CAD build for the part. Positions are in the model's coordinates, mm. A direction names the side the tool comes from. Coordinates: 2 decimals unless noted, no trailing zeros. Write each question's results on one line, items separated by ' | '.
from build123d import *

# Parameters (mm, degrees)
EXTRUDE_1_DEPTH     = 3
SKETCH_7_R          = 1
CUT_EXTRUDE_2_DEPTH = 6.5
FILLET_3_R          = 1
CUT_EXTRUDE_START   = -43.5
SKETCH_8_R          = 1.5
CUT_EXTRUDE_3_DEPTH = 51.446160402


with BuildPart() as part:
    # 草图4 for 放样1 → 放样1 section 0
    with BuildSketch(Plane(origin=(0, 80, 0), x_dir=(1, 0, 0), z_dir=(0, 1, 0))):
        with BuildLine():
            Line((-17.603437889, 42.498458496), (-16.455387592, 39.726819898))
            # circular arc as an exact rational Bezier (weights 1, cos(half-angle), 1)
            Bezier((-16.455387592, 39.726819898), (0, 46.542864613), (16.455387592, 39.726819898), weights=[1, 0.923879533, 1])
            Line((16.455387592, 39.726819898), (17.603437889, 42.498458496))
            Bezier((17.603437889, 42.498458496), (0, 49.790041213), (-17.603437889, 42.498458496), weights=[1, 0.923879533, 1])
        make_face()
    # 草图3 for 放样1 → 放样1 section 1
    with BuildSketch(Plane(origin=(0, 0, 0), x_dir=(1, 0, 0), z_dir=(0, 1, 0))):
        with BuildLine():
            Line((-17.603437889, 42.498458496), (-16.455387592, 39.726819898))
            Bezier((-16.455387592, 39.726819898), (0, 46.542864613), (16.455387592, 39.726819898), weights=[1, 0.923879533, 1])
            Line((16.455387592, 39.726819898), (17.603437889, 42.498458496))
            Bezier((17.603437889, 42.498458496), (0, 49.790041213), (-17.603437889, 42.498458496), weights=[1, 0.923879533, 1])
        make_face()
    loft()

    # 草图6 → 凸台-拉伸1 (add)
    with BuildSketch(Plane.XZ):
        with BuildLine():
            Line((-6.009200316, -42.57804025), (-6.009200316, -45.605805678))
            ThreePointArc((-6.009200316, -45.605805678), (-4.257725406, -45.802530218), (-2.5, -45.932014979))
            Line((-2.5, -45.932014979), (-2.5, -42.927264064))
            ThreePointArc((-2.5, -42.927264064), (-4.258181751, -42.788642046), (-6.009200316, -42.57804025))
        make_face()
        with BuildLine():
            ThreePointArc((2.5, -45.932014979), (4.257725406, -45.802530218), (6.009200316, -45.605805678))
            Line((6.009200316, -45.605805678), (6.009200316, -42.57804025))
            ThreePointArc((6.009200316, -42.57804025), (4.258181751, -42.788642046), (2.5, -42.927264064))
            Line((2.5, -42.927264064), (2.5, -45.932014979))
        make_face()
    extrude(amount=EXTRUDE_1_DEPTH)

    # 草图7 → 切除-拉伸2 (cut, symmetric)
    with BuildSketch(Plane(origin=(0, 0, 0), x_dir=(0, 0, -1), z_dir=(1, 0, 0))):
        with Locations((44.081332421, -1.518353576)):
            Circle(SKETCH_7_R)
    extrude(amount=CUT_EXTRUDE_2_DEPTH, both=True, mode=Mode.SUBTRACT)

    # 圆角3
    fillet_3_edges = [part.edges().sort_by_distance(p)[0] for p in [
        (4.257725406, -3, -45.802530218),
        (4.258181751, -3, -42.788642046),
        (-4.257725406, -3, -45.802530218),
        (-4.258181751, -3, -42.788642046),
    ]]
    fillet(fillet_3_edges, radius=FILLET_3_R)

    # 草图8 → 切除-拉伸3 (cut, through all)
    with BuildSketch(Plane.XY.offset(CUT_EXTRUDE_START)):
        with Locations((0, 40)):
            Circle(SKETCH_8_R)
    extrude(amount=-CUT_EXTRUDE_3_DEPTH, mode=Mode.SUBTRACT)


solid = part.part
1) Which spindle directions (+Z, -Z, +X, -X, +Y, -Y) get a long thin tool onto all of the face, cutting with end or side? Do faces 4 (the flat face through (-12, 0, -43)), 5 (the flat face through (12, 0, -43)), 6 (the flat face through (2.5, -0.8, -45.1)), 7 (the flat face through (0, 40, -43.5)), 8 (the cylindrical face through (4.283, -0.986, -42.786)). Say none if no direction does.
Outcome:
face 4: +Z, -Z, -X, -Y | face 5: +Z, -Z, +X, -Y | face 6: +Z, -Z, -Y | face 7: -Z | face 8: +Z, +Y, -Y
2) Two-plate mould, pull along Z, no slides. Class faces 1 (the cylindrical face through (-0.325, 38.536, -44.733)), 2 (the cylindrical face through (-4.23, -1.474, -43.082)), 3 (the cylindrical face through (-4.23, -0.99, -42.79)): pulls with the +Z half, pulls with the -Z half, needs draft (parallel to the pull), parting line crosses it, or undercut.
Outcome:
face 1: needs draft | face 2: undercut | face 3: pulls with the +Z half
3) Drill centre lines: L1, parallel to Y at x = 3, z = -44; L2, parallel to Y at x = 0, z = -44.6; L3, parallel to Y at x = -9.5, z = -43.25. Where is each one in solid material? Low to high. Write a range as from..to.
Outcome:
L1: y = -3..-2.52, -0.52..80 | L2: y = 0..38.5, 41.5..80 | L3: y = 0..80
4) Pin check, flat tips, straight feed: pin 1 (2 mm diameter, centred on x = 3.5, y = 19.5, fed in from -Z); pin 2 (1.5 mm diameter, centred on x = -0.5, y = 37.5, fed in from +Z); pin 3 (3 mm diameter, centred on x = 14, z = -41.5, fed in from -Y); pin 4 (1.6 mm diameter, centred on y = -1.52, z = -44.08, fed in from -X). Stop position of each tip, or through.
Outcome:
pin 1: stops at z = -45.93 | pin 2: stops at z = -42.98 | pin 3: stops at y = 0 | pin 4: passes through
